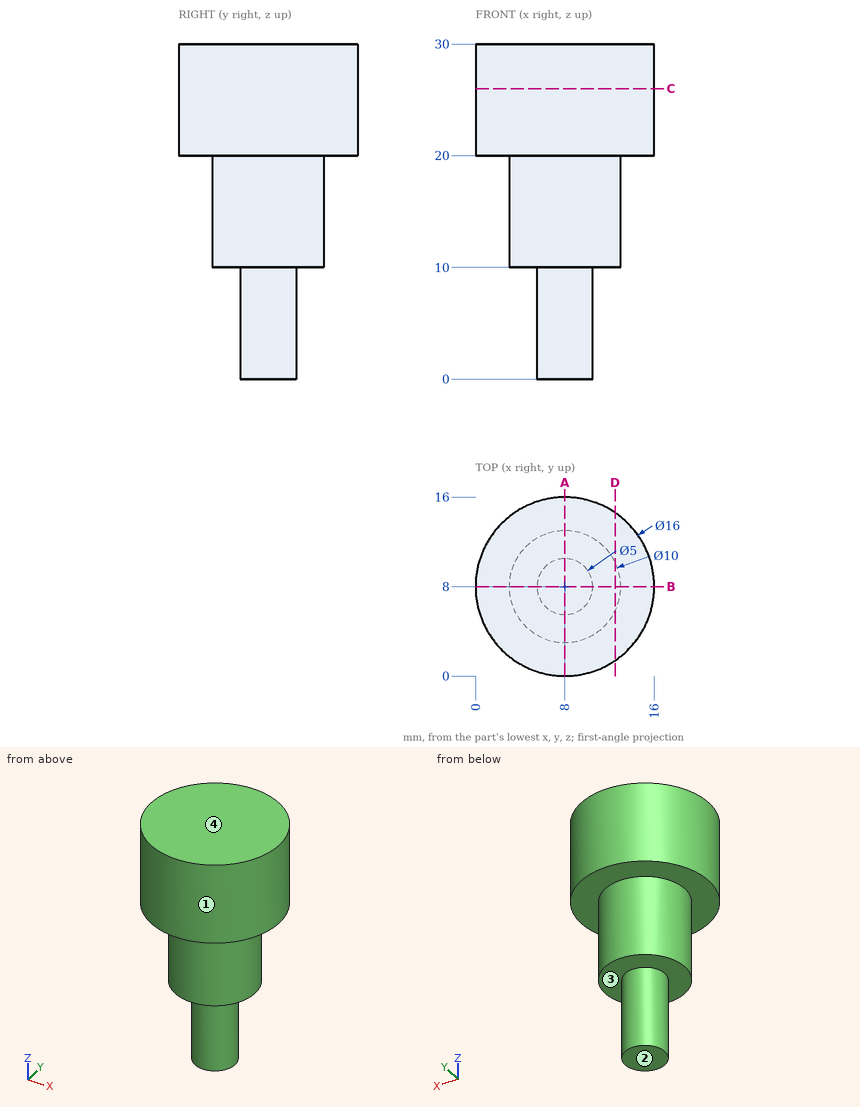
Answer from the drawing. Dimensions are ordinates in mm from the lowest x, y and z of the part. A direction names the side the tool comes from. Round coordinates to 2 decimals unless told otherwise and drop trailing zeros. Write each loop counter-clockwise with the first axis right and the second up, starting at its lowest first coordinate (ties: lowest second). Pieces come first, ordered by that corner, then holes. Notation, with made-up numbers: M 3.5,4.25 L 41.5,4.25 A14 cw 41.5,10.25 Z; hole C -4,-10 d6. An arc over 180 degrees is marked long. Write each question's results on one line, items separated by ' | '. Start each with the question number.
Item 1: The mould has two halves that part along X. Classify the marked faces 1 and 2: +X half, -X half, draft (parallel to the pull), parting line (faces both ways), or undercut.
Item 2: Which of the six approach directions +Z, -Z, +X, -X, +Y, -Y give full straight-line access (tool end or side, diameter ignored) to the marked faces 3 and 4?
Item 3: Straight lines are drawn through the part: probe 1 along Z at (x, y) = (2.75, 7.25); probe 2 along Z at (x, y) = (11.5, 8.5); probe 3 along Y at (x, z) = (11.5, 14.75). For each, find the intervals that lie inside material, in ascending order.
Item 4: Given pin 1 Ø1.5 at (x, y) = (9, 4) entering from -Z; pin 2 Ø6 at (x, y) = (8.5, 10.5) entering from -Z; pin 3 Ø5 at (x, z) = (6, 15) entering from +Y; pin 4 Ø2 at (y, z) = (13, 18.5) entering from -X, each flat-ended and moving along its own axis, determine where each tip first touches the part or whether it passes through.
Item 5: Find section D-D on x = 12.5. Write down the section's boundary in (y, z).
Item 6: Find section C-C on z = 26. Write down the section's boundary in (x, y).
Item 7: Find section A-A on x = 8. Write down the section's boundary in (y, z).
Answer block:
1) face 1: parting line | face 2: draft
2) face 3: -Z | face 4: +Z, +X, -X, +Y, -Y
3) probe 1: z = 20 to 30 | probe 2: z = 10 to 30 | probe 3: y = 4.43 to 11.57
4) pin 1: stops at z = 10 | pin 2: stops at z = 0 | pin 3: stops at y = 13 | pin 4: stops at x = 5
5) outline: M 1.39,20 L 5.82,20 L 5.82,10 L 10.18,10 L 10.18,20 L 14.61,20 L 14.61,30 L 1.39,30 Z
6) outline: C 8,8 d16
7) outline: M 0,20 L 3,20 L 3,10 L 5.5,10 L 5.5,0 L 10.5,0 L 10.5,10 L 13,10 L 13,20 L 16,20 L 16,30 L 0,30 Z
